```python
from build123d import *

# Parameters (mm, degrees)
SKETCH2_R           = 1.5
BOSS_EXTRUDE1_DEPTH = 3


with BuildPart() as part:
    # Sketch1 → Revolve1 (revolve)
    with BuildSketch(Plane.XY, mode=Mode.PRIVATE) as revolve1_sk:
        Polygon((40.368689296, 141), (33, 141), (33, 143), (19.5, 143), (19.5, 173.5), (15.5, 173.5), (15.5, 137.5), (29.304292175, 137.5), (40.368689296, 137.5), align=None)
    revolve(revolve1_sk.sketch.rotate(Axis((0, 0, 0), (0, 1, 0)), 90), axis=Axis((0, 0, 0), (0, 1, 0)))

    # Sketch2 → Boss-Extrude1 (add)
    with BuildSketch(Plane(origin=(0, 173.5, 0), x_dir=(1, 0, 0), z_dir=(0, 1, 0))):
        with Locations(Location((17.5, 0, 0), (0, 0, 270))):
            Circle(SKETCH2_R)
        with Locations(Location((-17.5, 0, 0), (0, 0, 270))):
            Circle(SKETCH2_R)
    extrude(amount=BOSS_EXTRUDE1_DEPTH)


solid = part.part
```
Check sheet for the modelled part. Datum: model origin and axes. Units: mm. A direction names the side the tool comes from. Coordinates: 2 decimals unless noted, no trailing zeros. Write each loop counter-clockwise with the first axis right and the second up, starting at its lowest first coordinate (ties: lowest second). Pieces come first, ordered by that corner, then holes. Notation, with made-up numbers: M 60.5,36.5 L 95.5,36.5 A29 ccw 95.5,75.5 Z; hole C -21.75,73.5 d5. An arc over 180 degrees is marked long. Write item = value, one per line. Start each with the question number.
1. Sectioned sample at D-D (z = 21). Record the cut outline in (x, y), then the cut area to 3 significant figures.
2. Sectioned sample at C-C (x = -4). Record the cut outline in (y, z).
3. Thickness scan on probe 1 along X at (y, z) = (148, 0); probe 2 along Y at (x, z) = (-19, -17.5); probe 3 along Z at (x, y) = (-12.5, 167). Record the ranges inside material, lowest first.
4. Sectioned sample at B-B (y = 174.5). Record the cut outline in (x, z).
5. Go/stop test with flat-tipped pins: pin 1 (18.5 mm diameter, centred on x = 0, z = 0, fed in from +Y); pin 2 (6 mm diameter, centred on x = -17, z = -28.5, fed in from +Y); pin 3 (1.5 mm diameter, centred on x = 2.5, z = -19.5, fed in from +Y); pin 4 (2 mm diameter, centred on x = 31.5, z = 23, fed in from +Y). Record where each tip stops, or that it passes through.
6. Mould release check, pull along X, two halves, no side actions. Record for faces 3 (the flat face through (-1, 137.5, 17)), 4 (the cylindrical face through (-15.368, 155.248, 2.018)), 5 (the cylindrical face through (-9.912, 142.014, -31.476)): pulls with the +X half, pulls with the -X half, needs draft (parallel to the pull), parting line crosses it, or undercut.
7. Tool access check on faces 1 (the flat face through (-17, 176.5, 0)), 2 (the cylindrical face through (-19.334, 158.464, 2.539)). Record the directions out of +Z, -Z, +X, -X, +Y, -Y that give a thin tool (end or side, any length) a straight path to the whole face; none if there is none.
8. Sectioned sample at A-A (z = 0). Record the cut outline in (x, y).
The answers:
q1.outline = M -34.48,137.5 L 34.48,137.5 L 34.48,141 L 25.46,141 L 25.46,143 L -25.46,143 L -25.46,141 L -34.48,141 Z
q1.area = 343 mm²
q2.outline = M 137.5,-40.17 L 141,-40.17 L 141,-32.76 L 143,-32.76 L 143,-19.09 L 173.5,-19.09 L 173.5,-14.97 L 137.5,-14.97 Z; M 137.5,14.97 L 173.5,14.97 L 173.5,19.09 L 143,19.09 L 143,32.76 L 141,32.76 L 141,40.17 L 137.5,40.17 Z
q3.probe_1 = -19.5 to -15.5, 15.5 to 19.5
q3.probe_2 = 137.5 to 143
q3.probe_3 = -14.97 to -9.17, 9.17 to 14.97
q4.outline = C -17.5,0 d3; C 17.5,0 d3
q5.pin_1 = through
q5.pin_2 = 143
q5.pin_3 = 173.5
q5.pin_4 = 141
q6.face_3 = needs draft
q6.face_4 = undercut
q6.face_5 = parting line crosses it
q7.face_1 = +Z, -Z, +X, -X, +Y
q7.face_2 = +Y
q8.outline = M -40.37,137.5 L -15.5,137.5 L -15.5,173.5 L -16,173.5 L -16,176.5 L -19,176.5 L -19,173.5 L -19.5,173.5 L -19.5,143 L -33,143 L -33,141 L -40.37,141 Z; M 15.5,137.5 L 40.37,137.5 L 40.37,141 L 33,141 L 33,143 L 19.5,143 L 19.5,173.5 L 19,173.5 L 19,176.5 L 16,176.5 L 16,173.5 L 15.5,173.5 Z
